from build123d import *

# Parameters (mm, degrees)
SKETCH1_R           = 165
SKETCH1_R_2         = 20
BOSS_EXTRUDE1_DEPTH = 15
CUT_EXTRUDE1_DEPTH  = 30
FILLET1_R           = 30
SKETCH3_R           = 4.5
CUT_EXTRUDE2_DEPTH  = 20


with BuildPart() as part:
    # Sketch1 → Boss-Extrude1 (new body)
    with BuildSketch(Plane.XY):
        Circle(SKETCH1_R)
        with Locations((0, 117)):
            Circle(SKETCH1_R_2, mode=Mode.SUBTRACT)
        with Locations((101.324972243, -58.5)):
            Circle(SKETCH1_R_2, mode=Mode.SUBTRACT)
        with Locations((-101.324972243, -58.5)):
            Circle(SKETCH1_R_2, mode=Mode.SUBTRACT)
    extrude(amount=BOSS_EXTRUDE1_DEPTH)

    # Sketch2 → Cut-Extrude1 (cut)
    with BuildSketch(Plane.XY.offset(15)):
        with BuildLine():
            Line((-38.302222156, -97.860619516), (-169.990854036, -254.801019663))
            Line((-169.990854036, -254.801019663), (115.890035572, -190.326174896))
            Line((115.890035572, -190.326174896), (38.302222156, -97.860619516))
            ThreePointArc((38.302222156, -97.860619516), (0, -80), (-38.302222156, -97.860619516))
        make_face()
        with BuildLine():
            Line((-65.598671453, 82.101007166), (-135.66872892, 274.616907838))
            Line((-135.66872892, 274.616907838), (-222.772320251, -5.200627403))
            Line((-222.772320251, -5.200627403), (-103.900893609, 15.759612349))
            ThreePointArc((-103.900893609, 15.759612349), (-69.282032303, 40), (-65.598671453, 82.101007166))
        make_face()
        with BuildLine():
            Line((103.900893609, 15.759612349), (305.659582957, -19.815888175))
            Line((305.659582957, -19.815888175), (106.882284679, 195.526802298))
            Line((106.882284679, 195.526802298), (65.598671453, 82.101007166))
            ThreePointArc((65.598671453, 82.101007166), (69.282032303, 40), (103.900893609, 15.759612349))
        make_face()
    extrude(amount=-CUT_EXTRUDE1_DEPTH, mode=Mode.SUBTRACT)

    # Fillet1
    fillet1_edges = [part.edges().sort_by_distance(p)[0] for p in [
        (164.924238662, 4.999550163, 7.5),
        (86.79185678, 140.328805299, 7.5),
        (-86.79185678, 140.328805299, 7.5),
        (-164.924238662, 4.999550163, 7.5),
        (-78.132381882, -145.328355463, 7.5),
        (78.132381882, -145.328355463, 7.5),
    ]]
    fillet(fillet1_edges, radius=FILLET1_R)

    # Sketch3 → Cut-Extrude2 (cut)
    with BuildSketch(Plane.XY.offset(15)):
        with Locations((0, 20)):
            Circle(SKETCH3_R)
        with Locations((17.320508076, -10)):
            Circle(SKETCH3_R)
        with Locations((-17.320508076, -10)):
            Circle(SKETCH3_R)
    extrude(amount=-CUT_EXTRUDE2_DEPTH, mode=Mode.SUBTRACT)


solid = part.part
Can you work these out from the model? Positions are in its coordinate system, mm. A direction names the side the tool comes from. Coordinates: 2 decimals unless noted, no trailing zeros. Order: outer loops, then holes, each group sorted by start corner. A loop starts at its lowest first (then second) coordinate and runs counter-clockwise, first axis right, second up. Notation, with made-up numbers: M 77.5,1 L 103.5,1 A14 cw 103.5,11 Z; hole C -35.75,60 d8. An arc over 180 degrees is marked long. Answer as CSV lines item,"result".
(1) Suppose I cut it at C-C on z = 9.5. Please give me the cut outline in (x, y), plus the area to 3 significant figures.
Geometry check:
outline,"M -163.19,-24.35 A165 ccw -102.69,-129.15 A30 ccw -61.04,-124.95 L -38.3,-97.86 A50 cw 38.3,-97.86 L 61.04,-124.95 A30 ccw 102.69,-129.15 A165 ccw 163.19,-24.35 A30 ccw 138.73,9.62 L 103.9,15.76 A50 cw 65.6,82.1 L 77.69,115.34 A30 ccw 60.51,153.51 A165 ccw -60.51,153.51 A30 ccw -77.69,115.34 L -65.6,82.1 A50 cw -103.9,15.76 L -138.73,9.62 A30 ccw Z; hole C -101.32,-58.5 d40; hole C -17.32,-10 d9; hole C 0,117 d40; hole C 0,20 d9; hole C 17.32,-10 d9; hole C 101.32,-58.5 d40"
area,"55,000 mm^2"
(2) I'm going to push flat-ended pins straight in: pin 1 (2 mm diameter, centred on y = -61, z = 3.5, fed in from -X); pin 2 (1 mm diameter, centred on x = -62.5, z = 9, fed in from +Y); pin 3 (5 mm diameter, centred on y = 74, z = 4, fed in from -X). Where does each tip first touch, or does it pass through?
Geometry check:
pin 1,"x = -153.7"
pin 2,"y = 152.87"
pin 3,"x = -63.92"
(3) Suppose I cut it at B-B on y = 122. Please give me the cut outline in (x, z), plus the area to 3 significant figures.
Geometry check:
outline,"M -79.29,0 L -19.36,0 L -19.36,15 L -79.29,15 Z; M 19.36,0 L 79.29,0 L 79.29,15 L 19.36,15 Z"
area,"1,800 mm^2"
(4) On a 3-axis mill with a long thin cutter (end or side, diameter ignored), from which of +Z, -Z, +X, -X, +Y, -Y can I reach the whole of each face in a straight line? I mean faces 5 (the flat face through (49.83, -111.6, 7.6)), 6 (the flat face through (71.73, 98.95, 7.6)), 7 (the flat face through (121.072, 12.732, 7.605)). Say none if no direction works.
Geometry check:
face 5,"+Z, -Z, -Y"
face 6,"+Z, -Z, +X"
face 7,"+Z, -Z, +X, +Y"
(5) If we mould it in two halves opening along Y, with no side actions, what happens to faces 1 (the cylindrical face through (-143.326, -81.748, 7.395)), 2 (the cylindrical face through (77, 137.6, 7.4)), 3 (the flat face through (-2, -17, 0)), 4 (the cylindrical face through (-76.724, 138.21, 7.395))? For each: released by +Y, released by -Y, zero draft, split by the parting line, or undercut.
Geometry check:
face 1,"released by -Y"
face 2,"undercut"
face 3,"zero draft"
face 4,"undercut"
(6) Please list where these lines run through material, in increasing order: L1, parallel to X at y = -72, z = 6.25; L2, parallel to X at y = -74.5, z = 3; L3, parallel to X at y = -86, z = 6.25.
Geometry check:
L1,"-148.46 to -116.08, -86.57 to 86.57, 116.08 to 148.46"
L2,"-147.22 to -113.32, -89.32 to 89.32, 113.32 to 147.22"
L3,"-140.82 to -23.75, 23.75 to 140.82"
(7) Suppose I cut it at D-D on y = -58.5. Please give me the cut outline in (x, z), plus the area to 3 significant figures.
Geometry check:
outline,"M -154.28,0 L -121.32,0 L -121.32,15 L -154.28,15 Z; M -81.32,0 L 81.32,0 L 81.32,15 L -81.32,15 Z; M 121.32,0 L 154.28,0 L 154.28,15 L 121.32,15 Z"
area,"3,430 mm^2"
(8) Suppose I cut it at A-A on x = 0. Please give me the cut outline in (y, z).
Geometry check:
outline,"M -80,0 L 15.5,0 L 15.5,15 L -80,15 Z; M 24.5,0 L 97,0 L 97,15 L 24.5,15 Z; M 137,0 L 165,0 L 165,15 L 137,15 Z"
